```python
from build123d import *

# Parameters (mm, degrees)
SKETCH_1_R      = 9
EXTRUDE_1_DEPTH = 10


with BuildPart() as part:
    # 草图1 → 凸台-拉伸1 (new body)
    with BuildSketch(Plane.XY):
        with Locations((-0.274924045, -0.151737187)):
            Circle(SKETCH_1_R)
        with BuildLine():
            Line((-4.274924045, 6.320398768), (3.725075955, 6.320398768))
            Line((3.725075955, 6.320398768), (3.725075955, 4.320398768))
            ThreePointArc((3.725075955, 4.320398768), (-0.274924045, -6.151737187), (-4.274924045, 4.320398768))
            Line((-4.274924045, 4.320398768), (-4.274924045, 6.320398768))
        make_face(mode=Mode.SUBTRACT)
    extrude(amount=EXTRUDE_1_DEPTH)


solid = part.part
```
Design review of the part built by this model. Coordinates are the model's own, in mm. A direction names the side the tool comes from. Round coordinates to 2 decimals unless told otherwise and drop trailing zeros. Write each loop counter-clockwise with the first axis right and the second up, starting at its lowest first coordinate (ties: lowest second). Pieces come first, ordered by that corner, then holes.
Item 1: We need section A-A on y = -2.75. Write out the cut boundary in (x, z).
Item 2: For probe 1 along X at (y, z) = (0, 3); probe 2 along X at (y, z) = (-3.5, 5.25); probe 3 along Y at (x, z) = (-1.75, 1), list the stretches that pass through material, from the lowest coordinate up.
Item 3: For faces 1 (the flat face through (3.725, 5, 5)), 2 (the flat face through (2, -6, 10)), list the 3-axis set-ups (+Z, -Z, +X, -X, +Y, -Y) from which the entire face can be reached by the end or side of a thin tool; tool diameter is ignored.
Item 4: We need section C-C on z = 6.25. Write out the cut boundary in (x, y).
Item 5: We need section B-B on x = -1. Write out the cut boundary in (y, z).
Item 6: We need section D-D on x = -7. Write out the cut boundary in (y, z).
Item 7: The part is to be moulded in two halves that separate along X. For faces 3 (the cylindrical face through (8.31, 2.55, 4.93)), 4 (the flat face through (2, -6, 0)), 5 (the flat face through (0, 6.32, 5)), say which applies: +X half, -X half, draft (parallel to the pull), parting line (faces both ways), or undercut.
Item 8: Clearance check with flat-ended pins moving along their axes: pin 1 Ø6 at (y, z) = (-4.5, 1) entering from -X; pin 2 Ø5 at (x, z) = (5, 3.5) entering from -Y; pin 3 Ø3 at (y, z) = (2, 6) entering from +X; pin 4 Ø5 at (y, z) = (0.5, 7.5) entering from -X. State where each tip first meets the part, or that it passes through.
Returned:
1. outline: (-8.89, 0) - (-5.68, 0) - (-5.68, 10) - (-8.89, 10) - close; (5.13, 0) - (8.34, 0) - (8.34, 10) - (5.13, 10) - close
2. probe 1: x = -9.27 to -6.27, 5.72 to 8.72
2. probe 2: x = -8.63 to -5.25, 4.7 to 8.08
2. probe 3: y = -9.03 to -5.97, 6.32 to 8.73
3. face 1: +Z, -Z
3. face 2: +Z, +X, -X, +Y, -Y
4. outline: circle Ø18 at (-0.27, -0.15); hole (-4.27, 4.32) arc R6 ccw (long way) to (3.73, 4.32) - (3.73, 6.32) - (-4.27, 6.32) - close
5. outline: (-9.12, 0) - (-6.11, 0) - (-6.11, 10) - (-9.12, 10) - close; (6.32, 0) - (8.82, 0) - (8.82, 10) - (6.32, 10) - close
6. outline: (-6.13, 0) - (5.83, 0) - (5.83, 10) - (-6.13, 10) - close
7. face 3: parting line
7. face 4: draft
7. face 5: undercut
8. pin 1: stops at x = -9.17
8. pin 2: stops at y = -8.71
8. pin 3: stops at x = 8.7
8. pin 4: stops at x = -9.27
